Verification items for the finished model (mm, model axes). Round coordinates to 2 decimals unless told otherwise and drop trailing zeros. Order: outer loops, then holes, each group sorted by start corner. A loop starts at its lowest first (then second) coordinate and runs counter-clockwise, first axis right, second up. Notation, with made-up numbers: M 30.5,84.5 L 71.5,84.5 A15 ccw 71.5,105.5 Z; hole C -35,7.5 d11. An arc over 180 degrees is marked long. Use CSV: the item, a comma, the result in double quotes. Start each with the question number.
Q1. Sectioned sample at B-B (z = 0). Enter the section's corners in (x, y), and give its area (3 significant figures).
Q2. Scan lines: line 1 (Z direction, x = -15.5, y = 0.9); line 2 (X direction, y = 1.3, z = 8.75); line 3 (X direction, y = 0.3, z = -16). Record each from-to range of solid material in increasing order.
Q3. Mould release check, pull along Z, two halves, no side actions. Record for faces 1 (the face through (-9, 3, 9)), 2 (the face through (-17.206, 1.479, 8.295)), 3 (the face through (6.31, 1.48, 20.03)): +Z half, -Z half, draft (parallel to the pull), parting line (faces both ways), or undercut.
Q4. Sectioned sample at C-C (z = 10). Enter the section's corners in (x, y).
Q5. Sectioned sample at D-D (y = 0.95). Enter the section's corners in (x, z), and give its area (3 significant figures).
Q6. Gauge pin test, flat ends, axial feed: pin 1 Ø4 at (x, z) = (-15.16, 8.75) entering from +Y; pin 2 Ø1 at (x, y) = (-9, 1) entering from +Z. Record the tip position at first contact, or that the pin passes through.
Q7. Sectioned sample at A-A (x = 0). Enter the section's corners in (y, z), and give its area (3 significant figures).
```python
from build123d import *

# Parameters (mm, degrees)
SKETCH_1_R      = 21
SKETCH_1_R_2    = 12.5
SKETCH_1_R_3    = 2.1
EXTRUDE_1_DEPTH = 3


with BuildPart() as part:
    # 草图1 → 凸台-拉伸1 (new body)
    with BuildSketch(Plane(origin=(0, 0, 0), x_dir=(1, 0, 0), z_dir=(0, 1, 0))):
        with Locations(Location((0, 0, 0), (0, 0, 270))):
            Circle(SKETCH_1_R)
        with Locations(Location((0, 0, 0), (0, 0, 270))):
            Circle(SKETCH_1_R_2, mode=Mode.SUBTRACT)
        with Locations(Location((0, 17.5, 0), (0, 0, 270))):
            Circle(SKETCH_1_R_3, mode=Mode.SUBTRACT)
        with Locations(Location((15.155444566, 8.75, 0), (0, 0, 270))):
            Circle(SKETCH_1_R_3, mode=Mode.SUBTRACT)
        with Locations(Location((15.155444566, -8.75, 0), (0, 0, 270))):
            Circle(SKETCH_1_R_3, mode=Mode.SUBTRACT)
        with Locations(Location((0, -17.5, 0), (0, 0, 270))):
            Circle(SKETCH_1_R_3, mode=Mode.SUBTRACT)
        with Locations(Location((-15.155444566, -8.75, 0), (0, 0, 270))):
            Circle(SKETCH_1_R_3, mode=Mode.SUBTRACT)
        with Locations(Location((-15.155444566, 8.75, 0), (0, 0, 270))):
            Circle(SKETCH_1_R_3, mode=Mode.SUBTRACT)
    extrude(amount=EXTRUDE_1_DEPTH)


solid = part.part
```
Verdict:
1,outline,"M -21,0 L -12.5,0 L -12.5,3 L -21,3 Z; M 12.5,0 L 21,0 L 21,3 L 12.5,3 Z"
1,area,"51.0 mm²"
2,line 1,"z = -14.17 to -10.82, -6.68 to 6.68, 10.82 to 14.17"
2,line 2,"x = -19.09 to -17.26, -13.06 to -8.93, 8.93 to 13.06, 17.26 to 19.09"
2,line 3,"x = -13.6 to -1.47, 1.47 to 13.6"
3,face 1,"draft"
3,face 2,"undercut"
3,face 3,"parting line"
4,outline,"M -18.47,0 L -16.84,0 L -16.84,3 L -18.47,3 Z; M -13.47,0 L -7.5,0 L -7.5,3 L -13.47,3 Z; M 7.5,0 L 13.47,0 L 13.47,3 L 7.5,3 Z; M 16.84,0 L 18.47,0 L 18.47,3 L 16.84,3 Z"
5,outline,"C 0,0 d42; hole C -15.16,-8.75 d4.2; hole C -15.16,8.75 d4.2; hole C 0,0 d25; hole C 0,-17.5 d4.2; hole C 0,17.5 d4.2; hole C 15.16,-8.75 d4.2; hole C 15.16,8.75 d4.2"
5,area,"811 mm²"
6,pin 1,"passes through"
6,pin 2,"stops at z = 19.2"
7,outline,"M 0,-21 L 3,-21 L 3,-19.6 L 0,-19.6 Z; M 0,-15.4 L 3,-15.4 L 3,-12.5 L 0,-12.5 Z; M 0,12.5 L 3,12.5 L 3,15.4 L 0,15.4 Z; M 0,19.6 L 3,19.6 L 3,21 L 0,21 Z"
7,area,"25.8 mm²"
